Read the model definition and answer for the solid it produces. Units are mm, in the model's axes. Face numbers are marked on the shaded views. A direction names the side the tool comes from. Give positions to 0.01 mm unless a question says otherwise; leave off trailing zeros. Order: outer loops, then holes, each group sorted by start corner. A loop starts at its lowest first (then second) coordinate and runs counter-clockwise, first axis right, second up. Notation, with made-up numbers: (52.5, -17) - (84.5, -17) arc R30 ccw to (84.5, 14) - close; hole circle Ø6 at (44, 25). An arc over 180 degrees is marked (long way). Write each question's results on one line, items separated by ' | '. Start each with the question number.
Q1. Find section C-C on z = 3.5. Give the vertices of the cut face in (x, y), and give its area (3 significant figures).
Q2. For a pull along Y with two mould halves and no side action, classify the marked faces 3, 4 and 5 as +Y half, -Y half, draft (parallel to the pull), parting line (faces both ways), or undercut.
Q3. Flat-ended cylindrical pins translate along their axes: P1, Ø2, axis at y = 4.5, z = -1, coming from the -X side; P2, Ø5, axis at x = -7.5, z = -2, coming from the -Y side; P3, Ø13, axis at x = -2.5, y = 0.5, coming from the -Z side; P4, Ø2, axis at y = 6.5, z = 4, coming from the +X side (3 decimals). Find the tip coordinate at first contact, or state that the pin passes through.
Q4. Find section D-D on z = -5. Give the vertices of the cut face in (x, y), and give its area (3 significant figures).
Q5. Find section A-A on x = 0. Give the vertices of the cut face in (y, z).
Q6. Find the intervals of material crossed by line 1 along Y through (x, z) = (0, -2.75); line 2 along Y through (x, z) = (0, 3.4); line 3 along Z through (x, y) = (-5.75, -2), in increasing order. Write a range as from..to.
Q7. A tool of negligible diameter and unlimited length cuts with its end or side. For the marked faces 1 and 2, from which of +Z, -Z, +X, -X, +Y, -Y can it reach the whole face along a straight path? Write none if from no direction.
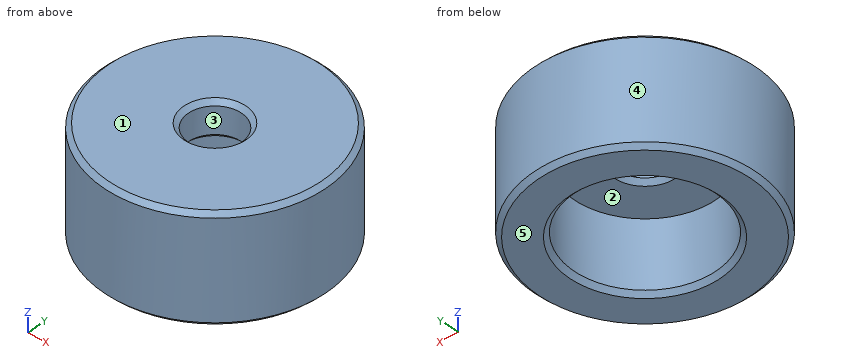
from build123d import *

# Parameters (mm, degrees)
SKETCH1_R           = 12.5
SKETCH1_R_2         = 3
BOSS_EXTRUDE1_DEPTH = 6
SKETCH2_R           = 8
CUT_EXTRUDE1_DEPTH  = 8
CHAMFER1_SIZE       = 0.5


with BuildPart() as part:
    # Sketch1 → Boss-Extrude1 (new, symmetric)
    with BuildSketch(Plane.XY):
        Circle(SKETCH1_R)
        Circle(SKETCH1_R_2, mode=Mode.SUBTRACT)
    extrude(amount=BOSS_EXTRUDE1_DEPTH, both=True)

    # Sketch2 → Cut-Extrude1 (cut)
    with BuildSketch(Plane(origin=(0, 0, -6), x_dir=(-1, 0, 0), z_dir=(0, 0, -1))):
        Circle(SKETCH2_R)
    extrude(amount=-CUT_EXTRUDE1_DEPTH, mode=Mode.SUBTRACT)

    # Chamfer1
    chamfer1_edges = [part.edges().sort_by_distance(p)[0] for p in [
        (-3, 0, 2),
        (8, 0, -6),
        (-12.5, 0, -6),
        (-12.5, 0, 6),
        (-3, 0, 6),
    ]]
    chamfer(chamfer1_edges, length=CHAMFER1_SIZE)


solid = part.part
Working result:
1) outline: circle Ø25 at (0, 0); hole circle Ø6 at (0, 0) | area: 463 mm²
2) face 3: undercut | face 4: parting line | face 5: draft
3) P1: x = -12 | P2: y = -11.46 | P3: z = -6 | P4: x = 11.225
4) outline: circle Ø25 at (0, 0); hole circle Ø16 at (0, 0) | area: 290 mm²
5) outline: (-12.5, -5.5) - (-12, -6) - (-8.5, -6) - (-8, -5.5) - (-8, 2) - (-3.5, 2) - (-3, 2.5) - (-3, 5.5) - (-3.5, 6) - (-12, 6) - (-12.5, 5.5) - close; (3, 2.5) - (3.5, 2) - (8, 2) - (8, -5.5) - (8.5, -6) - (12, -6) - (12.5, -5.5) - (12.5, 5.5) - (12, 6) - (3.5, 6) - (3, 5.5) - close
6) line 1: -12.5..-8, 8..12.5 | line 2: -12.5..-3, 3..12.5 | line 3: 2..6
7) face 1: +Z, +X, -X, +Y, -Y | face 2: -Z
